```python
from build123d import *

# Parameters (mm, degrees)
SKETCH_1_R      = 1.55
SKETCH_1_R_2    = 1.3
EXTRUDE_1_DEPTH = 3
SKETCH_2_W      = 0.25
SKETCH_2_H      = 13.633784975
EXTRUDE_2_DEPTH = 3
FILLET_R2_1_R   = 2
FILLET_R1_1_R   = 1


with BuildPart() as part:
    # 草图1 → 凸台-拉伸1 (new body)
    with BuildSketch(Plane(origin=(0, 0, 0), x_dir=(0, 0, -1), z_dir=(1, 0, 0))):
        with BuildLine():
            Line((-14.25, 6.116215025), (-9.25, 6.116215025))
            Line((-9.25, 6.116215025), (-9.25, 19.75))
            Line((-9.25, 19.75), (-19.25, 19.75))
            Line((-19.25, 19.75), (-19.25, 0))
            ThreePointArc((-19.25, 0), (-20.641242789, -3.358757211), (-24, -4.75))
            Line((-24, -4.75), (-25.4, -4.75))
            Line((-25.4, -4.75), (-25.4, -9.75))
            Line((-25.4, -9.75), (-24, -9.75))
            ThreePointArc((-24, -9.75), (-17.105708883, -6.894291117), (-14.25, 0))
            Line((-14.25, 0), (-14.25, 6.116215025))
        make_face()
        with Locations((-13, 15.75)):
            Circle(SKETCH_1_R, mode=Mode.SUBTRACT)
        with Locations((-16.75, 5.25)):
            Circle(SKETCH_1_R, mode=Mode.SUBTRACT)
        with Locations((-16.5, 11.05)):
            Circle(SKETCH_1_R_2, mode=Mode.SUBTRACT)
        with Locations((-21.4, -7.034912935)):
            Circle(SKETCH_1_R_2, mode=Mode.SUBTRACT)
        with Locations((-16.917350474, -2.466997302)):
            Circle(SKETCH_1_R, mode=Mode.SUBTRACT)
    extrude(amount=EXTRUDE_1_DEPTH)

    # 草图2 → 凸台-拉伸2 (add, through all)
    with BuildSketch(Plane(origin=(3, 0, 0), x_dir=(0, 0, -1), z_dir=(1, 0, 0))):
        with BuildLine():
            Line((-19.25, 19.75), (-11.75, 19.75))
            Line((-11.75, 19.75), (-11.75, 22.25))
            Line((-11.75, 22.25), (-12.576690734, 22.25))
            ThreePointArc((-12.576690734, 22.25), (-14.402080928, 22.212645368), (-13.5, 23.8))
            Line((-13.5, 23.8), (-13.5, 26.25))
            Line((-13.5, 26.25), (-21.2, 26.25))
            ThreePointArc((-21.2, 26.25), (-22.99246212, 25.50753788), (-22.25, 27.3))
            Line((-22.25, 27.3), (-22.25, 28.75))
            Line((-22.25, 28.75), (-25.25, 28.75))
            Line((-25.25, 28.75), (-25.25, 25.25))
            ThreePointArc((-25.25, 25.25), (-24.753426104, 22.95535741), (-23.352564103, 21.071330896))
            ThreePointArc((-23.352564103, 21.071330896), (-20.323673289, 16.997760056), (-19.25, 12.036370673))
            Line((-19.25, 12.036370673), (-19.25, 19.75))
        make_face()
        with Locations((-9.125, 12.933107513)):
            Rectangle(SKETCH_2_W, SKETCH_2_H)
    extrude(amount=-EXTRUDE_2_DEPTH)

    # R2 圆角1
    fillet_r2_1_edges = [part.edges().sort_by_distance(p)[0] for p in [
        (1.5, 6.116215025, 14.25),
    ]]
    fillet(fillet_r2_1_edges, radius=FILLET_R2_1_R)

    # R1 圆角1
    fillet_r1_1_edges = [part.edges().sort_by_distance(p)[0] for p in [
        (1.5, -9.75, 25.4),
        (1.5, 19.75, 11.75),
        (1.5, 19.75, 9),
        (1.5, 6.116215025, 9),
    ]]
    fillet(fillet_r1_1_edges, radius=FILLET_R1_1_R)


solid = part.part
```
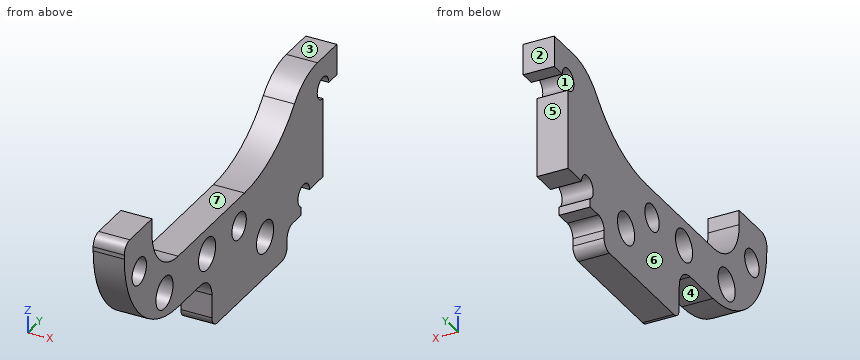
The listing builds one solid part. Answer for the finished solid, in the listing's coordinates (mm). Face numbers are marked on the shaded views. A direction names the side the tool comes from. Coordinates: 2 decimals unless noted, no trailing zeros. Write each loop counter-clockwise with the first axis right and the second up, starting at its lowest first coordinate (ties: lowest second). Pieces come first, ordered by that corner, then holes.
Q1. Section D-D, the plane x = 2 is taken. Give the number of separate pieces and of enclosed holes in the cut face, then the cut area to 3 significant figures.
Returned:
separate pieces: 1
enclosed holes: 5
area: 286 mm2
Q2. Given P1, Ø0.9, axis at x = 1, y = 3, coming from the -Z side; P2, Ø0.7, axis at x = 1.5, z = 11, coming from the -Y side; P3, Ø0.7, axis at x = 2, y = 25, coming from the -Z side, each flat-ended and moving along its own axis, determine where each tip first touches the part or whether it passes through.
Returned:
P1: stops at z = 14.25
P2: stops at y = 6.12
P3: stops at z = 13.5
Q3. Section C-C, the plane z = 13 is taken. Write down the section's boundary in (x, y), then the cut area to 3 significant figures.
Returned:
outline: (0, 5.97) - (3, 5.97) - (3, 14.2) - (0, 14.2) - close; (0, 17.3) - (3, 17.3) - (3, 21.83) - (0, 21.83) - close
area: 38.3 mm2
Q4. The mould has two halves that part along Y. Classify the marked faces 1, 2 and 3: released by +Y, released by -Y, zero draft, split by the parting line, or undercut.
Returned:
face 1: undercut
face 2: released by +Y
face 3: zero draft
Q5. Which of the six approach directions +Z, -Z, +X, -X, +Y, -Y give full straight-line access (tool end or side, diameter ignored) to the marked faces 4, 5, 6 and 7?
Returned:
face 4: -Z, +X, -X, -Y
face 5: -Z, +X, -X, +Y
face 6: +Z, -Z, -X, +Y, -Y
face 7: +Z, +X, -X
Q6. Section A-A, the plane y = 11.05 is taken. Write down the section's boundary in (x, z), then the cut area to 4 significant figures.
Returned:
outline: (0, 9) - (3, 9) - (3, 15.2) - (0, 15.2) - close; (0, 17.8) - (3, 17.8) - (3, 19.25) - (0, 19.25) - close
area: 22.95 mm2
Q7. Section B-B, the plane z = 16.75 is taken. Write down the section's boundary in (x, y).
Returned:
outline: (0, -6.52) - (3, -6.52) - (3, -4.01) - (0, -4.01) - close; (0, -0.93) - (3, -0.93) - (3, 3.7) - (0, 3.7) - close; (0, 6.8) - (3, 6.8) - (3, 9.77) - (0, 9.77) - close; (0, 12.33) - (3, 12.33) - (3, 26.25) - (0, 26.25) - close
Q8. Find the intervals of material crossed by line 1 along Y through (x, z) = (2.8, 21.5); line 2 along Y through (x, z) = (0.8, 16.5); line 3 along Y through (x, z) = (1.1, 15.5), in increasing order.
Returned:
line 1: y = -9.42 to -8.33, -5.74 to -4.04, 19.03 to 25.52
line 2: y = -6.23 to -3.96, -0.97 to 3.72, 6.78 to 9.75, 12.35 to 26.25
line 3: y = -4.78 to -3.09, -1.84 to 4.33, 6.17 to 10.22, 11.88 to 26.25
